Check sheet for the modelled part. Datum: model origin and axes. Units: mm. Round coordinates to 2 decimals unless told otherwise and drop trailing zeros. Loops run counter-clockwise (first coordinate to the right, second up) from the corner with the lowest first, then second, coordinate; pieces in that order, holes last. Notation, with made-up numbers: (70.25, 41) -> (91.25, 41) arc R36 cw to (91.25, 77) -> close; hole circle Ø3 at (36.25, -39). An arc over 180 degrees is marked (long way). One line per question, with ' | ' between items.
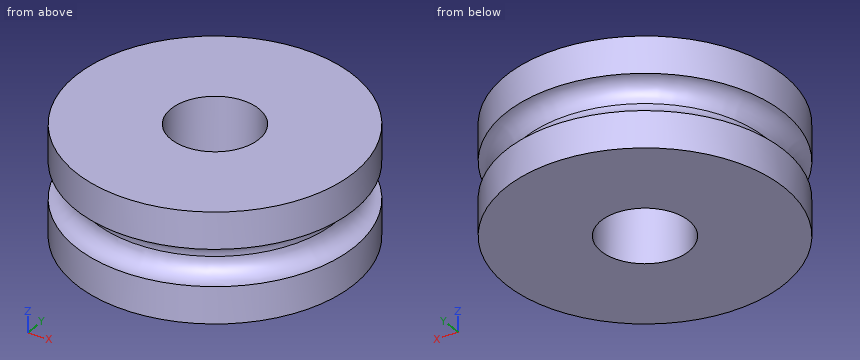
```python
from build123d import *

# Parameters (mm, degrees)
SKETCH1_R           = 38
SKETCH1_R_2         = 12
BOSS_EXTRUDE1_DEPTH = 30
SKETCH2_R           = 5


with BuildPart() as part:
    # Sketch1 → Boss-Extrude1 (new body)
    with BuildSketch(Plane.XY):
        Circle(SKETCH1_R)
        Circle(SKETCH1_R_2, mode=Mode.SUBTRACT)
    extrude(amount=BOSS_EXTRUDE1_DEPTH)

    # Sketch2 → Cut-Revolve1 (revolve, cut)
    with BuildSketch(Plane(origin=(0, 0, 0), x_dir=(1, 0, 0), z_dir=(0, 1, 0))):
        with Locations((-38, -15)):
            Circle(SKETCH2_R)
    revolve(axis=Axis((0, 0, 0), (0, 0, 1)), mode=Mode.SUBTRACT)


solid = part.part
```
(1) Sectioned sample at D-D, the plane z = 13.25. Record the cut outline in (x, y).
Answer:
outline: circle Ø66.63 at (0, 0); hole circle Ø24 at (0, 0)
(2) Sectioned sample at C-C, the plane z = 3. Record the cut outline in (x, y), and give its area (3 significant figures).
Answer:
outline: circle Ø76 at (0, 0); hole circle Ø24 at (0, 0) | area: 4,080 mm2
(3) Go/stop test with flat-tipped pins: pin 1 (8 mm diameter, centred on y = -26, z = 4, fed in from +X); pin 2 (1.5 mm diameter, centred on y = 13.5, z = 10.5, fed in from +X); pin 3 (3 mm diameter, centred on x = 16, z = 3.5, fed in from +Y). Record where each tip stops, or that it passes through.
Answer:
pin 1: stops at x = 30.98 | pin 2: stops at x = 35.73 | pin 3: stops at y = 35.12
(4) Scan lines: probe 1 along Y at (x, z) = (0, 22); probe 2 along Z at (x, y) = (0, 34); probe 3 along Z at (x, y) = (20, -29). Record each from-to range of solid material in increasing order.
Answer:
probe 1: y = -38 to -12, 12 to 38 | probe 2: z = 0 to 12, 18 to 30 | probe 3: z = 0 to 10.84, 19.16 to 30
(5) Sectioned sample at A-A, the plane x = 0. Record the cut outline in (y, z).
Answer:
outline: (-38, 0) -> (-12, 0) -> (-12, 30) -> (-38, 30) -> (-38, 20) arc R5 cw to (-38, 10) -> close; (12, 0) -> (38, 0) -> (38, 10) arc R5 cw to (38, 20) -> (38, 30) -> (12, 30) -> close
